The model under review builds one solid part; all positions refer to its coordinate system, in mm. Face numbers are marked on the shaded views. A direction names the side the tool comes from. Give positions to 0.01 mm unless a question says otherwise; leave off trailing zeros. Order: outer loops, then holes, each group sorted by start corner. A loop starts at its lowest first (then second) coordinate and runs counter-clockwise, first axis right, second up. Notation, with made-up numbers: (-23.75, 83) - (19.25, 83) arc R27 ccw to (19.25, 115) - close; hole circle Ø3 at (82.25, 10). An arc over 180 degrees is marked (long way). Use a Markdown table: item, result. Add a question column.
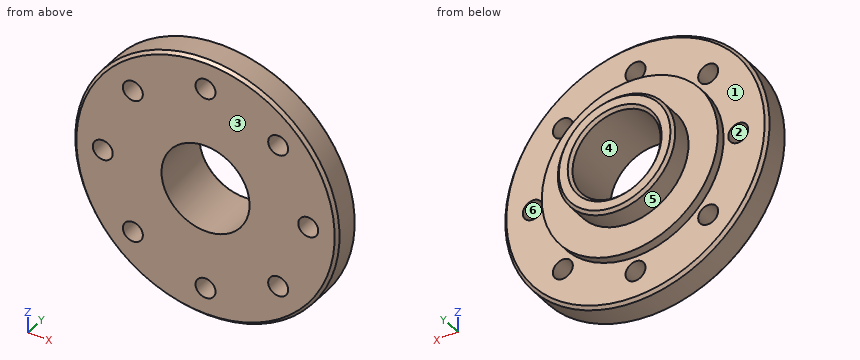
```python
from build123d import *

# Parameters (mm, degrees)
SKETCH1_R           = 20
BOSS_EXTRUDE1_DEPTH = 8
SKETCH3_R           = 30
BOSS_EXTRUDE2_DEPTH = 3
SKETCH4_R           = 45
BOSS_EXTRUDE3_DEPTH = 10
SKETCH5_R           = 15
CUT_EXTRUDE1_DEPTH  = 60
M8_TAPPED_HOLE1_D   = 6.8
CIRPATTERN2_COUNT   = 8
CHAMFER1_SIZE       = 1
CHAMFER2_SIZE       = 1


with BuildPart() as part:
    # Sketch1 → Boss-Extrude1 (new body)
    with BuildSketch(Plane(origin=(0, 0, 0), x_dir=(1, 0, 0), z_dir=(0, 1, 0))):
        with Locations(Location((0, 0, 0), (0, 0, 270))):
            Circle(SKETCH1_R)
    extrude(amount=BOSS_EXTRUDE1_DEPTH)

    # Sketch3 → Boss-Extrude2 (add)
    with BuildSketch(Plane.XZ):
        with Locations(Location((0, 0, 0), (0, 0, 270))):
            Circle(SKETCH3_R)
    extrude(amount=BOSS_EXTRUDE2_DEPTH)

    # Sketch4 → Boss-Extrude3 (add)
    with BuildSketch(Plane.XZ.offset(3)):
        with Locations(Location((0, 0, 0), (0, 0, 270))):
            Circle(SKETCH4_R)
    extrude(amount=BOSS_EXTRUDE3_DEPTH)

    # Sketch5 → Cut-Extrude1 (cut)
    with BuildSketch(Plane(origin=(0, 8, 0), x_dir=(1, 0, 0), z_dir=(0, 1, 0))):
        with Locations(Location((0, 0, 0), (0, 0, 270))):
            Circle(SKETCH5_R)
    extrude(amount=-CUT_EXTRUDE1_DEPTH, mode=Mode.SUBTRACT)

    # M8 Tapped Hole1 (through all)
    with Locations(Plane(origin=(0, -13, 0), x_dir=(-1, 0, 0), z_dir=(0, -1, 0))):
        with Locations((0, -35)):
            m8_tapped_hole1 = Hole(M8_TAPPED_HOLE1_D / 2)

    # CirPattern2: M8 Tapped Hole1 ×8 about axis
    cirpattern2_axis = Axis((0, 0, 0), (0, 1, 0))
    for i in range(1, CIRPATTERN2_COUNT):
        add(m8_tapped_hole1.rotate(cirpattern2_axis, i * 360 / CIRPATTERN2_COUNT), mode=Mode.SUBTRACT)

    # Chamfer1
    chamfer1_edges = [part.edges().sort_by_distance(p)[0] for p in [
        (0, -13, 45),
        (0, -3, 45),
    ]]
    chamfer(chamfer1_edges, length=CHAMFER1_SIZE)

    # Chamfer2
    chamfer2_edges = [part.edges().sort_by_distance(p)[0] for p in [
        (0, 8, -15),
        (0, 8, -20),
    ]]
    chamfer(chamfer2_edges, length=CHAMFER2_SIZE)


solid = part.part
```
Q1. We need section C-C (y = -1.5). Write out the cut boundary in (x, z).
Q2. We need section A-A (z = 0). Count the separate pieces of the cut face and the enclosed holes in it, plus the area to 3 significant figures.
Q3. Wall thickness on probe 1 along X at (y, z) = (-5, 0); probe 2 along X at (y, z) = (-4.25, 24.5); probe 3 along X at (y, z) = (2, 0): over which ranges is each line inside the solid? List them lowest first.
Q4. Draft analysis for pull direction X (two halves, no side actions). For the marked faces 3, 4, 5 and 6, state which applies: pulls with the +X half, pulls with the -X half, needs draft (parallel to the pull), parting line crosses it, or undercut.
Q5. Machinability: for the marked faces 1 and 2, which of the approach directions +Z, -Z, +X, -X, +Y, -Y give a long, thin tool a straight path to every point of the face, cutting with its end or side? Answer none if there is none.
Q6. Clearance check with flat-ended pins moving along their axes: P1, Ø2, axis at y = -8.5, z = -24, coming from the -X side; P2, Ø1, axis at x = -35.5, z = -27.5, coming from the -Y side; P3, Ø12, axis at x = -2.5, y = 3.5, coming from the +Z side; P4, Ø8, axis at x = 0, z = 35, coming from the -Y side. State where each tip first meets the part, or that it passes through.
Here are the results:
| question | item | result |
|---|---|---|
| 1 | outline | circle Ø60 at (0, 0); hole circle Ø30 at (0, 0) |
| 2 | separate pieces | 4 |
| 2 | enclosed holes | 0 |
| 2 | area | 630 mm2 |
| 3 | probe 1 | -45 to -38.4, -31.6 to -15, 15 to 31.6, 38.4 to 45 |
| 3 | probe 2 | -37.75 to -28.14, -21.36 to 21.36, 28.14 to 37.75 |
| 3 | probe 3 | -20 to -15, 15 to 20 |
| 4 | face 3 | needs draft |
| 4 | face 4 | undercut |
| 4 | face 5 | parting line crosses it |
| 4 | face 6 | undercut |
| 5 | face 1 | +Y |
| 5 | face 2 | +Y, -Y |
| 6 | P1 | x = -38.68 |
| 6 | P2 | y = -12.59 |
| 6 | P3 | z = 30 |
| 6 | P4 | y = -13 |
